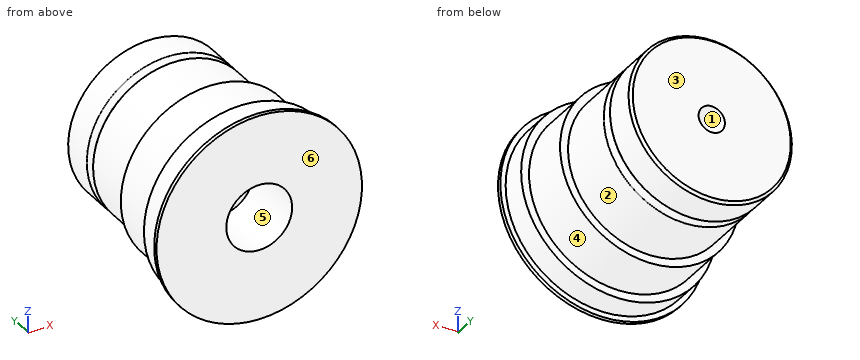
from build123d import *

# Parameters (mm, degrees)
CHAMFER_1_SIZE = 1


with BuildPart() as part:
    # 草图1 → 旋转1 (revolve)
    with BuildSketch(Plane.XY, mode=Mode.PRIVATE) as revolve_1_sk:
        with BuildLine():
            Line((-12.5, 0), (-12.5, 25))
            Line((-12.5, 25), (-5, 25))
            Line((-5, 25), (-5, 71.5))
            Line((-5, 71.5), (-31, 71.5))
            Line((-31, 71.5), (-31, 58.624264069))
            ThreePointArc((-31, 58.624264069), (-30.97716386, 58.509459039), (-30.912132034, 58.412132034))
            Line((-30.912132034, 58.412132034), (-29.212132034, 56.712132034))
            ThreePointArc((-29.212132034, 56.712132034), (-29.124264069, 56.5), (-29.212132034, 56.287867966))
            Line((-29.212132034, 56.287867966), (-30.912132034, 54.587867966))
            ThreePointArc((-30.912132034, 54.587867966), (-30.97716386, 54.490540961), (-31, 54.375735931))
            Line((-31, 54.375735931), (-31, 31.5))
            Line((-31, 31.5), (-34, 31.5))
            Line((-34, 31.5), (-34, 11.5))
            Line((-34, 11.5), (-37, 11.5))
            Line((-37, 11.5), (-37, 1.5))
            Line((-37, 1.5), (-39, 1.5))
            Line((-39, 1.5), (-39, 0))
            Line((-39, 0), (-12.5, 0))
        make_face()
    revolve(revolve_1_sk.sketch.rotate(Axis((0, 0, 0), (0, 1, 0)), 270), axis=Axis((0, 0, 0), (0, 1, 0)))

    # 倒角1
    chamfer_1_edges = [part.edges().sort_by_distance(p)[0] for p in [
        (0, 71.5, 31),
    ]]
    chamfer(chamfer_1_edges, length=CHAMFER_1_SIZE)


solid = part.part
CAD build for the part. Positions are in the model's coordinates, mm. Face numbers are marked on the shaded views. A direction names the side the tool comes from. Round coordinates to 2 decimals unless told otherwise and drop trailing zeros. Write each loop counter-clockwise with the first axis right and the second up, starting at its lowest first coordinate (ties: lowest second). Pieces come first, ordered by that corner, then holes.
(1) Drop flat-ended pins along their axis: P1, Ø13, axis at x = 0, z = 0, coming from the -Y side; P2, Ø6, axis at x = -1.5, y = 10, coming from the +Z side; P3, Ø1.5, axis at x = 22, y = 54, coming from the -Z side. Give the stop position or say it passes through.
(2) 3-axis set-ups, long thin cutter, end or side, ignore diameter. For the marked faces 4, 5 and 6: which of +Z, -Z, +X, -X, +Y, -Y reach the whole face in a straight line?
(3) Probe line 1 along X through (y, z) = (60, 0); line 2 along X through (y, z) = (17.25, 0); line 3 along Y through (x, z) = (21, -21). List the from-to ranges inside material, lowest first.
(4) Mould opens along Z. For the marked faces 1, 2 and 3 say: pulls with the +Z half, pulls with the -Z half, needs draft (parallel to the pull), parting line crosses it, or undercut.
(5) Slice it at B-B, the plane y = 41. Write the cut outline in (x, z).
(6) Slice it at A-A, the plane y = 17. Write the cut outline in (x, z), and give its area (3 significant figures).
From the geometry:
1. P1: stops at y = 25
1. P2: stops at z = 37
1. P3: stops at z = -22.57
2. face 4: +Y
2. face 5: -Y
2. face 6: +Z, -Z, +X, -X, -Y
3. line 1: x = -31 to -5, 5 to 31
3. line 2: x = -34 to -12.5, 12.5 to 34
3. line 3: y = 0 to 55.8, 57.2 to 71.5
4. face 1: undercut
4. face 2: parting line crosses it
4. face 3: needs draft
5. outline: circle Ø62 at (0, 0); hole circle Ø10 at (0, 0)
6. outline: circle Ø68 at (0, 0); hole circle Ø25 at (0, 0)
6. area: 3,140 mm2
